```python
from build123d import *

# Parameters (mm, degrees)
SKETCH1_R                    = 825
SKETCH1_R_2                  = 500
BOSS_EXTRUDE1_DEPTH          = 25
F_24_5_24_5_DIAMETER_HOLE1_D = 26


with BuildPart() as part:
    # Sketch1 → Boss-Extrude1 (new body)
    with BuildSketch(Plane(origin=(0, 0, 0), x_dir=(1, 0, 0), z_dir=(0, 1, 0))):
        with Locations(Location((0, 0, 0), (0, 0, 270))):
            Circle(SKETCH1_R)
        with Locations(Location((0, 0, 0), (0, 0, 270))):
            Circle(SKETCH1_R_2, mode=Mode.SUBTRACT)
    extrude(amount=BOSS_EXTRUDE1_DEPTH)

    # Ø24.5 (24.5) Diameter Hole1 (through all)
    with Locations(Plane(origin=(0, 25, 0), x_dir=(1, 0, 0), z_dir=(0, 1, 0))):
        with Locations((0, 775), (134.577337692, 763.226008584), (265.065611077, 728.261781109), (387.5, 671.169687933), (548.00775542, 548.00775542), (634.842834324, 444.521738172), (702.388534953, 327.529152849), (748.592515374, 200.584759954), (775, 0), (763.226008584, -134.577337692), (728.261781109, -265.065611077), (671.169687933, -387.5), (548.00775542, -548.00775542), (444.521738172, -634.842834324), (327.529152849, -702.388534953), (200.584759954, -748.592515374), (0, -775), (-134.577337692, -763.226008584), (-265.065611077, -728.261781109), (-387.5, -671.169687933), (-548.00775542, -548.00775542), (-634.842834324, -444.521738172), (-702.388534953, -327.529152849), (-748.592515374, -200.584759954), (-775, 0), (-763.226008584, 134.577337692), (-728.261781109, 265.065611077), (-671.169687933, 387.5), (-548.00775542, 548.00775542), (-444.521738172, 634.842834324), (-327.529152849, 702.388534953), (-200.584759954, 748.592515374)):
            Hole(F_24_5_24_5_DIAMETER_HOLE1_D / 2)


solid = part.part
```
The listing builds one solid part. Answer for the finished solid, in the listing's coordinates (mm). Give positions to 0.01 mm unless a question says otherwise; leave off trailing zeros. Loops run counter-clockwise (first coordinate to the right, second up) from the corner with the lowest first, then second, coordinate; pieces in that order, holes last. Notation, with made-up numbers: (7, 80.25) - (65, 80.25) arc R11 ccw to (65, 95.25) - close; hole circle Ø10 at (0.25, -21.5). An arc over 180 degrees is marked (long way). Return JSON: item names as keys, results as strings. Group by question number.
1. Straight lines are drawn through the part: line 1 (Z direction, x = -204.5, y = 22.25); line 2 (X direction, y = 20.75, z = 328); line 3 (X direction, y = 1.5, z = -337). For each, find the intervals that lie inside material, in ascending order. Write a range as [from, to].
2. Find section A-A (z = -92). Write down the section's boundary in (x, y), then the cut area to 3 significant figures.
3. Given pin 1 Ø10 at (x, y) = (593.5, 12.5) entering from +Z; pin 2 Ø5 at (x, y) = (-561.5, 10.5) entering from +Z; pin 3 Ø10 at (x, y) = (411, 18.5) entering from +Z; pin 4 Ø1 at (x, z) = (609, -453) entering from -Y, each flat-ended and moving along its own axis, determine where each tip first touches the part or whether it passes through.
4. Determine the mould class of faces 1 (the cylindrical face through (247.808, 12.325, 786.903)), 2 (the cylindrical face through (21.984, 12.325, -499.516)), 3 (the flat face through (-355, 25, 355)) for opening direction Z: pulls with the +Z half, pulls with the -Z half, needs draft (parallel to the pull), parting line crosses it, or undercut.
5. Find section B-B (y = 20.75). State how many separate pieces and enclosed holes the cut face has, then the cut area to 3 significant figures.
Verdict:
{
 "1": {"line 1": "z = [-799.25, -760.99], [-736.2, -456.27], [456.27, 799.25]", "line 2": "x = [-756.99, -715.38], [-689.4, -377.38], [377.38, 756.99]", "line 3": "x = [-753.03, -369.37], [369.37, 693.48], [711.29, 753.03]"},
 "2": {"outline": "(-819.85, 0) - (-491.46, 0) - (-491.46, 25) - (-819.85, 25) - close; (491.46, 0) - (819.85, 0) - (819.85, 25) - (491.46, 25) - close", "area": "16,400 mm^2"},
 "3": {"pin 1": "stops at z = 578.18", "pin 2": "stops at z = 606.75", "pin 3": "stops at z = 718.18", "pin 4": "stops at y = 0"},
 "4": {"face 1": "parting line crosses it", "face 2": "undercut", "face 3": "needs draft"},
 "5": {"separate pieces": "1", "enclosed holes": "33", "area": "1,340,000 mm^2"}
}
